from build123d import *

# Parameters (mm, degrees)
ANGLED_BRACKET_BODY_DEPTH   = 20
GUIDE_UPRIGHT_BOSS_DEPTH    = 10
GUIDE_NOTCH_15X15_REACH     = 99.269
GUIDE_NOTCH_SKETCH_W        = 15
GUIDE_NOTCH_SKETCH_H        = 15
GUIDE_SLOTS_REACH           = 111.999
ANGLED_TRIM_CUT_45DEG_DEPTH = 96.535099634


with BuildPart() as part:
    # Bracket Profile Sketch → Angled Bracket Body (new, symmetric)
    with BuildSketch(Plane.XY):
        with BuildLine():
            Line((0, 5), (0, 30))
            Line((0, 30), (-10, 30))
            Line((-10, 30), (-10, 10))
            Line((-10, 10), (-64.142135624, 10))
            Line((-64.142135624, 10), (-85.355339059, -11.213203436))
            Line((-85.355339059, -11.213203436), (-78.284271247, -18.284271247))
            Line((-78.284271247, -18.284271247), (-60, 0))
            Line((-60, 0), (-5, 0))
            ThreePointArc((-5, 0), (-1.464466094, 1.464466094), (0, 5))
        make_face()
    extrude(amount=ANGLED_BRACKET_BODY_DEPTH, both=True)

    # Guide Upright Sketch → Guide Upright Boss (add)
    with BuildSketch(Plane(origin=(-37.071067812, 37.071067812, 0), x_dir=(0, 0, 1), z_dir=(-0.7071067811865486, 0.7071067811865465, 0))):
        with BuildLine():
            Line((-20, -68.284271247), (20, -68.284271247))
            ThreePointArc((20, -68.284271247), (0, -88.284271247), (-20, -68.284271247))
        make_face()
    extrude(amount=-GUIDE_UPRIGHT_BOSS_DEPTH)

    # Guide Notch Sketch → Guide Notch 15x15 (cut, up to next)
    with BuildSketch(Plane.ZY.offset(10), mode=Mode.PRIVATE) as guide_notch_15x15_sk1:
        with Locations((0, 22.5)):
            Rectangle(GUIDE_NOTCH_SKETCH_W, GUIDE_NOTCH_SKETCH_H)
    guide_notch_15x15_tool1 = extrude(guide_notch_15x15_sk1.sketch, amount=-GUIDE_NOTCH_15X15_REACH, mode=Mode.PRIVATE) & part.part
    add(guide_notch_15x15_tool1.solids().sort_by_distance((-10, 22.5, 0))[0], mode=Mode.SUBTRACT)

    # Guide Slots Sketch → Guide Slots (cut, up to next)
    with BuildSketch(Plane(origin=(0, 10, 0), x_dir=(1, 0, 0), z_dir=(0, 1, 0)), mode=Mode.PRIVATE) as guide_slots_sk1:
        with BuildLine():
            Line((-45, 15), (-25, 15))
            ThreePointArc((-25, 15), (-20, 10), (-25, 5))
            Line((-25, 5), (-45, 5))
            ThreePointArc((-45, 5), (-50, 10), (-45, 15))
        make_face()
    guide_slots_tool1 = extrude(guide_slots_sk1.sketch, amount=-GUIDE_SLOTS_REACH, mode=Mode.PRIVATE) & part.part
    # Guide Slots Sketch → Guide Slots (cut, up to next)
    with BuildSketch(Plane(origin=(0, 10, 0), x_dir=(1, 0, 0), z_dir=(0, 1, 0)), mode=Mode.PRIVATE) as guide_slots_sk2:
        with BuildLine():
            Line((-45, -15), (-25, -15))
            ThreePointArc((-25, -15), (-20, -10), (-25, -5))
            Line((-25, -5), (-45, -5))
            ThreePointArc((-45, -5), (-50, -10), (-45, -15))
        make_face()
    guide_slots_tool2 = extrude(guide_slots_sk2.sketch, amount=-GUIDE_SLOTS_REACH, mode=Mode.PRIVATE) & part.part
    add(guide_slots_tool1.solids().sort_by_distance((-35, 10, -10))[0], mode=Mode.SUBTRACT)
    add(guide_slots_tool2.solids().sort_by_distance((-35, 10, 10))[0], mode=Mode.SUBTRACT)

    # Angled Trim Sketch → Angled Trim Cut 45deg (cut, through all)
    with BuildSketch(Plane(origin=(-37.071067812, 37.071067812, 0), x_dir=(0, 0, 1), z_dir=(-0.7071067811865486, 0.7071067811865465, 0))):
        with BuildLine():
            Line((6.892487085, -78.712292238), (12.91897827, -84.738783423))
            Line((12.91897827, -84.738783423), (16.464043435, -81.212780777))
            Line((16.464043435, -81.212780777), (10.428020991, -75.176758332))
            ThreePointArc((10.428020991, -75.176758332), (-8.838834765, -59.445436483), (6.892487085, -78.712292238))
        make_face()
    extrude(amount=-ANGLED_TRIM_CUT_45DEG_DEPTH, mode=Mode.SUBTRACT)


solid = part.part
Could you check a few things on this model? Use its own coordinates, in mm. A direction names the side the tool comes from. Give positions to 0.01 mm unless a question says otherwise; leave off trailing zeros. Order: outer loops, then holes, each group sorted by start corner. A loop starts at its lowest first (then second) coordinate and runs counter-clockwise, first axis right, second up. Notation, with made-up numbers: (64.25, 35.5) - (104.25, 35.5) arc R15 ccw to (104.25, 55.5) - close; hole circle Ø3 at (15, 55.5). An arc over 180 degrees is marked (long way). One line per question, with ' | ' between items. Start each with the question number.
Item 1: I want a section at B-B on z = -0.5. Write out the boundary of the cut face in (x, y), then the cut area to 3 significant figures.
Item 2: I want a section at D-D on x = -15. Write out the boundary of the cut face in (y, z), then the cut area to 3 significant figures.
Item 3: I want a section at A-A on y = 17. Write out the boundary of the cut face in (x, z), then the cut area to 3 significant figures.
Item 4: I need wall thicknesses on probe 1 along Z at (x, y) = (-49, 9.5); probe 2 along Z at (x, y) = (-78, -8); probe 3 along X at (y, z) = (6, -6.5). Which ranges of each line are inside material? Lowest first, please. Write a range as [from, to].
Item 5: I want a section at C-C on z = -10. Write out the boundary of the cut face in (x, y), then the cut area to 3 significant figures.
Item 6: For faces 4 (the flat face through (-37, 10, 0)), 5 (the cylindrical face through (-20, 5, -10)), 6 (the flat face through (-33, 0, 0)), 7 (the flat face through (-5, 22, -7.5)), which set-ups out of +Z, -Z, +X, -X, +Y, -Y let a thin tool reach every point of the face, with its end or its side?
Item 7: Thinking about a two-plate mould opening in X: for faces 1 (the cylindrical face through (-50, 5, -10)), 2 (the flat face through (-5, 30, -14)), 3 (the flat face through (-10, 13, 0)), which applies, pulls with the +X half, pulls with the -X half, needs draft (parallel to the pull), parting line crosses it, or undercut?
Item 8: I'm going to push flat-ended pins straight in: pin 1 Ø20 at (x, z) = (-36, -3.5) entering from +Y; pin 2 Ø1 at (y, z) = (-4, -3.5) entering from -X; pin 3 Ø4 at (y, z) = (-10.5, 3.5) entering from -X. Where does each tip first touch, or does it pass through?
Verdict:
1) outline: (-99.49, -25.35) - (-92.42, -32.42) - (-87.12, -27.12) - (-94.19, -20.04) - close; (-76.52, -2.38) - (-69.45, -9.45) - (-60, 0) - (-5, 0) arc R5 ccw to (0, 5) - (0, 15) - (-10, 15) - (-10, 10) - (-64.14, 10) - close | area: 895 mm^2
2) outline: (0, -20) - (10, -20) - (10, 20) - (0, 20) - close | area: 400 mm^2
3) outline: (-10, -20) - (0, -20) - (0, -7.5) - (-10, -7.5) - close; (-10, 7.5) - (0, 7.5) - (0, 20) - (-10, 20) - close | area: 250 mm^2
4) probe 1: [-20, -13], [-7, 7], [13, 20] | probe 2: [-20, -10.02], [10.02, 20] | probe 3: [-68.14, -48.57], [-21.43, 0]
5) outline: (-97.6, -23.46) - (-90.53, -30.53) - (-83.59, -23.59) - (-90.66, -16.52) - close; (-80.05, -5.91) - (-72.98, -12.98) - (-60, 0) - (-50, 0) - (-50, 10) - (-64.14, 10) - close; (-20, 0) - (-5, 0) arc R5 ccw to (0, 5) - (0, 30) - (-10, 30) - (-10, 10) - (-20, 10) - close | area: 818 mm^2
6) face 4: +Z, -Z, -X, +Y | face 5: +Y, -Y | face 6: +Z, -Z, +X, -Y | face 7: +X, -X, +Y
7) face 1: undercut | face 2: needs draft | face 3: pulls with the -X half
8) pin 1: y = 10 | pin 2: x = -76.14 | pin 3: x = -71.31
